Can you work these out from the model? Positions are in its coordinate system, mm. Face numbers are marked on the shaded views. Coordinates: 2 decimals unless noted, no trailing zeros. Order: outer loops, then holes, each group sorted by start corner. A loop starts at its lowest first (then second) coordinate and runs counter-clockwise, first axis right, second up. Notation, with made-up numbers: (11, -7.5) -> (26, -7.5) arc R22 ccw to (26, 15.5) -> close; hole circle Ø11 at (76.25, 70.25). An arc over 180 degrees is marked (long way). Use a Markdown table: item, result. Add a question column.
1. Suppose I cut it at C-C, the plane x = 22. List the corners of the cut face in (y, z) for me.
2. We'd pull the mould along X, two halves only. Please class the marked faces 1, 2 and 3: pulls with the +X half, pulls with the -X half, needs draft (parallel to the pull), parting line crosses it, or undercut.
3. If I drill on line 1 along Y through (x, z) = (-28, 22); line 2 along Y through (x, z) = (28, 18.5); line 3 along X through (y, z) = (-6, 13), over which ranges is the centre line in solid material (lowest first)? Write a range as from..to.
4. For pin 1 Ø5 at (x, z) = (-93, 13) entering from +Y; pin 2 Ø1.5 at (y, z) = (160, 8.5) entering from +X; pin 3 Ø8 at (x, z) = (-79, 15.5) entering from -Y; pin 4 Ø10 at (x, y) = (-162.5, 125) entering from -Z, each with a flat end and sliding along its axis, tell me the tip position at first contact or that it passes through.
5. Suppose I cut it at D-D, the plane y = 62. List the corners of the cut face in (x, z) for me.
6. Suppose I cut it at A-A, the plane z = 7. List the corners of the cut face in (x, y) for me.
7. Suppose I cut it at B-B, the plane y = 0. List the corners of the cut face in (x, z) for me.
```python
from build123d import *

# Parameters (mm, degrees)
SKETCH1_R           = 38
BOSS_EXTRUDE1_DEPTH = 25


with BuildPart() as part:
    # Sketch1 → Boss-Extrude1 (new body)
    with BuildSketch(Plane.XY):
        with BuildLine():
            Line((-203, 198), (-203, -44.5))
            Line((-203, -44.5), (-193, -44.5))
            Line((-193, -44.5), (-193, -84.5))
            Line((-193, -84.5), (5.958881534, -66.734486818))
            ThreePointArc((5.958881534, -66.734486818), (66.949661999, -2.596682146), (11.109877523, 66.072464926))
            ThreePointArc((11.109877523, 66.072464926), (-55.326905119, 89.868640022), (-109.363154487, 135.257931614))
            ThreePointArc((-109.363154487, 135.257931614), (-151.670232074, 173.361739233), (-203, 198))
        make_face()
        Circle(SKETCH1_R, mode=Mode.SUBTRACT)
    extrude(amount=BOSS_EXTRUDE1_DEPTH)


solid = part.part
```
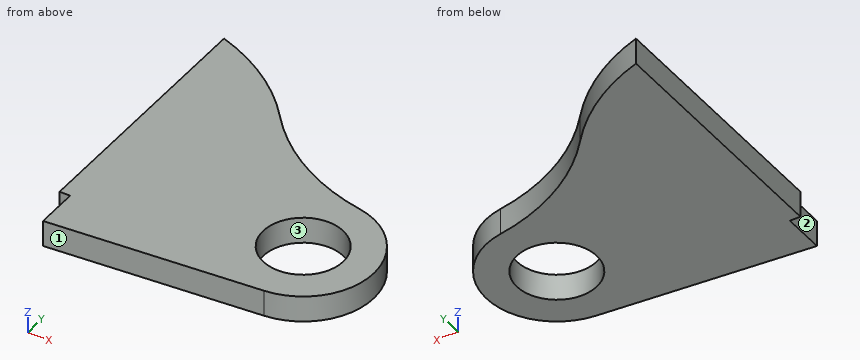
Worked out:
| question | item | result |
|---|---|---|
| 1 | outline | (-63.29, 0) -> (-30.98, 0) -> (-30.98, 25) -> (-63.29, 25) -> close; (30.98, 0) -> (63.29, 0) -> (63.29, 25) -> (30.98, 25) -> close |
| 2 | face 1 | pulls with the +X half |
| 2 | face 2 | pulls with the -X half |
| 2 | face 3 | undercut |
| 3 | line 1 | y = -69.77..-25.69, 25.69..76.82 |
| 3 | line 2 | y = -60.87..-25.69, 25.69..60.87 |
| 3 | line 3 | x = -203..-37.52, 37.52..66.73 |
| 4 | pin 1 | stops at y = 120.25 |
| 4 | pin 2 | stops at x = -133.06 |
| 4 | pin 3 | stops at y = -74.68 |
| 4 | pin 4 | stops at z = 0 |
| 5 | outline | (-203, 0) -> (25.4, 0) -> (25.4, 25) -> (-203, 25) -> close |
| 6 | outline | (-203, -44.5) -> (-193, -44.5) -> (-193, -84.5) -> (5.96, -66.73) arc R67 ccw to (11.11, 66.07) arc R200 cw to (-109.36, 135.26) arc R200 ccw to (-203, 198) -> close; hole circle Ø76 at (0, 0) |
| 7 | outline | (-203, 0) -> (-38, 0) -> (-38, 25) -> (-203, 25) -> close; (38, 0) -> (67, 0) -> (67, 25) -> (38, 25) -> close |
